from build123d import *

# Parameters (mm, degrees)
SKETCH3_R              = 12
CUT_EXTRUDE1_DEPTH     = 327.387806145
CIRPATTERN1_COUNT      = 6
SKETCH4_R              = 3
CUT_EXTRUDE5_DEPTH     = 327.387806145
CIRPATTERN2_COUNT      = 4
SKETCH5_R              = 130
CUT_EXTRUDE6_DEPTH     = 22
SKETCH6_R              = 175
CUT_EXTRUDE7_DEPTH     = 2
CHAMFER2_SIZE          = 2
CHAMFER2_SIZE2         = 1.154700538
CHAMFER3_SIZE          = 1
F_7_8_9_TAPPED_HOLE1_D = 19.44624
CIRPATTERN4_COUNT      = 2


with BuildPart() as part:
    # Sketch1 → Revolve1 (revolve)
    with BuildSketch(Plane.XY, mode=Mode.PRIVATE) as revolve1_sk:
        Polygon((0, 111), (0, 230), (-10, 230), (-10, 190), (-27, 190), (-27, 111), align=None)
    revolve(revolve1_sk.sketch.rotate(Axis((-73.563127278, 0, 0), (1, 0, 0)), 90), axis=Axis((-73.563127278, 0, 0), (1, 0, 0)))

    # Sketch3 → Cut-Extrude1 (cut, through all)
    with BuildSketch(Plane(origin=(0, 0, 0), x_dir=(0, 0, -1), z_dir=(1, 0, 0))):
        with Locations((-210, 0)):
            Circle(SKETCH3_R)
    cut_extrude1 = extrude(amount=-CUT_EXTRUDE1_DEPTH, mode=Mode.SUBTRACT)

    # CirPattern1: Cut-Extrude1 ×6 about axis
    cirpattern1_axis = Axis((0, 0, 0), (1, 0, 0))
    for i in range(1, CIRPATTERN1_COUNT):
        add(cut_extrude1.rotate(cirpattern1_axis, i * 360 / CIRPATTERN1_COUNT), mode=Mode.SUBTRACT)

    # Sketch4 → Cut-Extrude5 (cut, through all)
    with BuildSketch(Plane(origin=(0, 0, 0), x_dir=(0, 0, -1), z_dir=(1, 0, 0))):
        with Locations((-126, 0)):
            Circle(SKETCH4_R)
    cut_extrude5 = extrude(amount=-CUT_EXTRUDE5_DEPTH, mode=Mode.SUBTRACT)

    # CirPattern2: Cut-Extrude5 ×4 about axis
    cirpattern2_axis = Axis((0, 0, 0), (1, 0, 0))
    for i in range(1, CIRPATTERN2_COUNT):
        add(cut_extrude5.rotate(cirpattern2_axis, i * 360 / CIRPATTERN2_COUNT), mode=Mode.SUBTRACT)

    # Sketch5 → Cut-Extrude6 (cut)
    with BuildSketch(Plane.ZY.offset(27)):
        Circle(SKETCH5_R)
    extrude(amount=-CUT_EXTRUDE6_DEPTH, mode=Mode.SUBTRACT)

    # Sketch6 → Cut-Extrude7 (cut)
    with BuildSketch(Plane.ZY.offset(27)):
        Circle(SKETCH6_R)
    extrude(amount=-CUT_EXTRUDE7_DEPTH, mode=Mode.SUBTRACT)

    # Chamfer2
    chamfer2_edges = [part.edges().sort_by_distance(p)[0] for p in [
        (-25, 0, -130),
    ]]
    chamfer2_side = [part.faces().sort_by_distance(p)[0] for p in [
        (-15, 0, -130),
    ]]
    chamfer(chamfer2_edges, length=CHAMFER2_SIZE, length2=CHAMFER2_SIZE2, reference=chamfer2_side[0])

    # Chamfer3
    chamfer3_edges = [part.edges().sort_by_distance(p)[0] for p in [
        (0, 0, -230),
        (-27, 0, -190),
        (-10, 0, -230),
    ]]
    chamfer(chamfer3_edges, length=CHAMFER3_SIZE)

    # 7/8-9 Tapped Hole1 (through all)
    with Locations(Plane(origin=(0, 148.492424572, 148.492423527), x_dir=(0, 0, 1), z_dir=(1, 0, 0))):
        with Locations((0, 0)):
            f_7_8_9_tapped_hole1 = Hole(F_7_8_9_TAPPED_HOLE1_D / 2)

    # CirPattern4: 7/8-9 Tapped Hole1 ×2 about axis
    cirpattern4_axis = Axis((0, 0, 0), (1, 0, 0))
    for i in range(1, CIRPATTERN4_COUNT):
        add(f_7_8_9_tapped_hole1.rotate(cirpattern4_axis, i * 360 / CIRPATTERN4_COUNT), mode=Mode.SUBTRACT)


solid = part.part
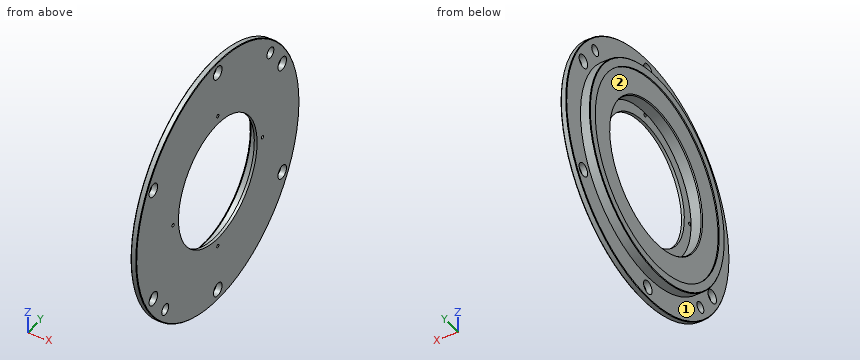
Design review of the part built by this model. Coordinates are the model's own, in mm. Face numbers are marked on the shaded views. Coordinates: 2 decimals unless noted, no trailing zeros. Order: outer loops, then holes, each group sorted by start corner. A loop starts at its lowest first (then second) coordinate and runs counter-clockwise, first axis right, second up. Notation, with made-up numbers: (83, 89.25) -> (128, 89.25) arc R20 cw to (128, 98.25) -> close; hole circle Ø8 at (28, -19.5). An arc over 180 degrees is marked (long way). Use one line per item in the form item = value. Start each with the question number.
(1) Add section A-A on x = -17.75. State the section outline as (y, z) points.
(2) Insertion check: pin 1 (1.5 mm diameter, centred on x = -12, y = -30.5, fed in from -Z); pin 2 (21.5 mm diameter, centred on y = -181.87, z = -105, fed in from +X); pin 3 (1 mm diameter, centred on x = -10, y = -9.5, fed in from -Z); pin 4 (22.5 mm diameter, centred on y = 148.49, z = 148.49, fed in from +X). Each pin has a flat end and moves straight along its axis. Give the tip position at first contact, or say it passes through.
(3) The part is to be moulded in two halves that separate along Z. For the marked faces 1 and 2, say which applies: +Z half, -Z half, draft (parallel to the pull), parting line (faces both ways), or undercut.
(4) For probe 1 along Z at (x, y) = (-3.25, -186); probe 2 along Y at (x, z) = (-12, 0); probe 3 along Z at (x, y) = (-1.1, -126), list the stretches that pass through material, from the lowest coordinate up.
Answer block:
q1.outline = circle Ø380 at (0, 0); hole circle Ø260 at (0, 0)
q2.pin_1 = -187.66
q2.pin_2 = through
q2.pin_3 = -229.3
q2.pin_4 = 0
q3.face_1 = draft
q3.face_2 = undercut
q4.probe_1 = -135.29 to -116.27, -93.73 to 93.73, 116.27 to 135.29
q4.probe_2 = -190 to -130, 130 to 190
q4.probe_3 = -192.42 to -3, 3 to 192.42
